Check sheet for the modelled part. Datum: model origin and axes. Units: mm. A direction names the side the tool comes from. Give positions to 0.01 mm unless a question says otherwise; leave off trailing zeros. Write each loop counter-clockwise with the first axis right and the second up, starting at its lowest first coordinate (ties: lowest second). Pieces come first, ordered by that corner, then holes. Notation, with made-up numbers: (54, -2) -> (77, -2) arc R13 cw to (77, 4) -> close; hole circle Ø2 at (70.5, 13.5). An arc over 180 degrees is marked (long way). Return JSON: item names as keys, results as strings.
from build123d import *

# Parameters (mm, degrees)
SKETCH_1_R          = 30.147889755
SKETCH_1_R_2        = 20.85
EXTRUDE_1_DEPTH     = 1.5
SKETCH_2_R          = 22.1
SKETCH_2_R_2        = 20.85
EXTRUDE_2_DEPTH     = 3.5
CHAMFER_C0_5_1_SIZE = 0.5
CHAMFER_2_SIZE      = 0.5
CHAMFER_2_SIZE2     = 1.866025404


with BuildPart() as part:
    # 草图1 → 凸台-拉伸1 (new body)
    with BuildSketch(Plane(origin=(0, 0, 0), x_dir=(1, 0, 0), z_dir=(0, 1, 0))):
        with Locations(Location((0, 0, 0), (0, 0, 270))):
            Circle(SKETCH_1_R)
        with Locations(Location((0, 0, 0), (0, 0, 270))):
            Circle(SKETCH_1_R_2, mode=Mode.SUBTRACT)
    extrude(amount=EXTRUDE_1_DEPTH)

    # 草图2 → 凸台-拉伸2 (add)
    with BuildSketch(Plane(origin=(0, 1.5, 0), x_dir=(1, 0, 0), z_dir=(0, 1, 0))):
        with Locations(Location((0, 0, 0), (0, 0, 270))):
            Circle(SKETCH_2_R)
        with Locations(Location((0, 0, 0), (0, 0, 270))):
            Circle(SKETCH_2_R_2, mode=Mode.SUBTRACT)
    extrude(amount=EXTRUDE_2_DEPTH)

    # C0.5 倒角1
    chamfer_c0_5_1_edges = [part.edges().sort_by_distance(p)[0] for p in [
        (0, 5, -22.1),
    ]]
    chamfer(chamfer_c0_5_1_edges, length=CHAMFER_C0_5_1_SIZE)

    # 倒角2
    chamfer_2_edges = [part.edges().sort_by_distance(p)[0] for p in [
        (0, 0, -30.147889755),
    ]]
    chamfer_2_side = [part.faces().sort_by_distance(p)[0] for p in [
        (0, 0.75, -30.147889755),
    ]]
    chamfer(chamfer_2_edges, length=CHAMFER_2_SIZE, length2=CHAMFER_2_SIZE2, reference=chamfer_2_side[0])


solid = part.part
(1) Cross-section at C-C on y = 2.9. Enter the section's corners in (x, z).
Reply:
{"outline": "circle Ø44.2 at (0, 0); hole circle Ø41.7 at (0, 0)"}
(2) Set-up check for faces 1 (the cylindrical face through (29.89, 0.99, -3.92)), 2 (the flat face through (16, 1.5, -16)): record each of +Z, -Z, +X, -X, +Y, -Y from which the full face is reachable in a straight line by a thin tool's end or side.
Reply:
{"face 1": "+Y, -Y", "face 2": "+Y"}
(3) Cross-section at B-B on z = 0. Enter the section's corners in (x, y), then the cut area to 3 significant figures.
Reply:
{"outline": "(-30.15, 0.5) -> (-28.28, 0) -> (-20.85, 0) -> (-20.85, 5) -> (-21.6, 5) -> (-22.1, 4.5) -> (-22.1, 1.5) -> (-30.15, 1.5) -> close; (20.85, 0) -> (28.28, 0) -> (30.15, 0.5) -> (30.15, 1.5) -> (22.1, 1.5) -> (22.1, 4.5) -> (21.6, 5) -> (20.85, 5) -> close", "area": "35.5 mm^2"}
(4) Thickness scan on L1, parallel to X at y = 1.65, z = 0; L2, parallel to X at y = 1.05, z = 17; L3, parallel to Z at x = -4.5, y = 4.65. Record the ranges inside material, lowest first.
Reply:
{"L1": "-22.1 to -20.85, 20.85 to 22.1", "L2": "-24.9 to -12.07, 12.07 to 24.9", "L3": "-21.48 to -20.36, 20.36 to 21.48"}
(5) Cross-section at A-A on x = 0. Enter the section's corners in (y, z).
Reply:
{"outline": "(0, -28.28) -> (0.5, -30.15) -> (1.5, -30.15) -> (1.5, -22.1) -> (4.5, -22.1) -> (5, -21.6) -> (5, -20.85) -> (0, -20.85) -> close; (0, 20.85) -> (5, 20.85) -> (5, 21.6) -> (4.5, 22.1) -> (1.5, 22.1) -> (1.5, 30.15) -> (0.5, 30.15) -> (0, 28.28) -> close"}
(6) Release check for a two-part mould opening along Z. For faces 3 (the cylindrical face through (-21.574, 2.979, -4.791)), 4 (the flat face through (18, 5, -11)), 5 (the cylindrical face through (20.673, 2.465, -2.714)) record: pulls with the +Z half, pulls with the -Z half, needs draft (parallel to the pull), parting line crosses it, or undercut.
Reply:
{"face 3": "parting line crosses it", "face 4": "needs draft", "face 5": "undercut"}
(7) Depth check by flat-ended pin: pin 1 Ø1 at (x, y) = (-10.5, 1) entering from -Z; pin 2 Ø3 at (x, y) = (17.5, 1) entering from -Z. Enter the tip coordinate at first touch or a pass-through.
Reply:
{"pin 1": "z = -28.44", "pin 2": "z = -25.55"}
